```python
from build123d import *

# Parameters (mm, degrees)
SKETCH_1_R               = 210
EXTRUDE_1_DEPTH          = 25
SKETCH_2_R               = 95.82
CUT_EXTRUDE_1_DEPTH      = 154
EXTRUDE_START            = 200
SKETCH_3_R               = 155.82
SKETCH_3_R_2             = 95.82
EXTRUDE_2_DEPTH          = 200
CHAMFER_1_SIZE           = 1
SKETCH_7_R               = 140.82
SKETCH_7_R_2             = 105.82
CUT_EXTRUDE_3_DEPTH      = 200
PATTERN_CIRCULAR_2_COUNT = 8


with BuildPart() as part:
    # 草图1 → 凸台-拉伸1 (new body)
    with BuildSketch(Plane(origin=(0, 0, 0), x_dir=(1, 0, 0), z_dir=(0, 1, 0))):
        with Locations(Location((0, 0, 0), (0, 0, 270))):
            Circle(SKETCH_1_R)
    extrude(amount=EXTRUDE_1_DEPTH)

    # 草图2 → 切除-拉伸1 (cut)
    with BuildSketch(Plane(origin=(0, 25, 0), x_dir=(1, 0, 0), z_dir=(0, 1, 0))):
        with Locations(Location((0, 0, 0), (0, 0, 270))):
            Circle(SKETCH_2_R)
    extrude(amount=-CUT_EXTRUDE_1_DEPTH, mode=Mode.SUBTRACT)

    # 草图3 → 凸台-拉伸2 (add)
    with BuildSketch(Plane(origin=(0, 25, 0), x_dir=(1, 0, 0), z_dir=(0, 1, 0)).offset(EXTRUDE_START)):
        with Locations(Location((0, 0, 0), (0, 0, 270))):
            Circle(SKETCH_3_R)
        with Locations(Location((0, 0, 0), (0, 0, 270))):
            Circle(SKETCH_3_R_2, mode=Mode.SUBTRACT)
    extrude(amount=-EXTRUDE_2_DEPTH)

    # 倒角1
    chamfer_1_edges = [part.edges().sort_by_distance(p)[0] for p in [
        (0, 225, -155.82),
        (0, 225, -95.82),
        (0, 0, -210),
        (0, 25, -210),
    ]]
    chamfer(chamfer_1_edges, length=CHAMFER_1_SIZE)

    # 草图7 → 切除-拉伸3 (cut)
    with BuildSketch(Plane(origin=(0, 225, 0), x_dir=(1, 0, 0), z_dir=(0, 1, 0))):
        with Locations(Location((0, 0, 0), (0, 0, 270))):
            Circle(SKETCH_7_R)
        with Locations(Location((0, 0, 0), (0, 0, 270))):
            Circle(SKETCH_7_R_2, mode=Mode.SUBTRACT)
    extrude(amount=-CUT_EXTRUDE_3_DEPTH, mode=Mode.SUBTRACT)

    # 草图10 → M10 六角圆柱头螺钉的柱形沉头孔2 (revolve, cut)
    with BuildSketch(Plane(origin=(-184.987401502, 25, 2.159001035), x_dir=(0, 0, 1), z_dir=(1, 0, 0))):
        Polygon((0, 0), (0, 30.804733405), (5.5, 27.5), (5.5, 11), (9, 11), (9, 0.025), (9.025, 0), align=None)
    hole_wizard_m10_2 = revolve(axis=Axis((-184.987401502, 31.35, 2.159001035), (0, -1, 0)), mode=Mode.SUBTRACT)

    # 阵列(圆周)2: M10 六角圆柱头螺钉的柱形沉头孔2 ×8 about axis
    pattern_circular_2_axis = Axis((0, 0, 0), (0, 1, 0))
    for i in range(1, PATTERN_CIRCULAR_2_COUNT):
        add(hole_wizard_m10_2.rotate(pattern_circular_2_axis, i * 360 / PATTERN_CIRCULAR_2_COUNT), mode=Mode.SUBTRACT)


solid = part.part
```
Source: CAD feature listing. Evaluate the final solid. Frame: model axes, mm. A direction names the side the tool comes from. Give positions to 0.01 mm unless a question says otherwise; leave off trailing zeros. Order: outer loops, then holes, each group sorted by start corner. A loop starts at its lowest first (then second) coordinate and runs counter-clockwise, first axis right, second up. Notation, with made-up numbers: (78.25, 75.25) -> (111.25, 75.25) arc R25 cw to (111.25, 112.25) -> close; hole circle Ø11 at (77, -22.75). An arc over 180 degrees is marked (long way). Use a Markdown table: item, result.
Q1. Section A-A (y = 104). Return the cut outline in (x, z), and give its area (3 significant figures).
A:
| item | result |
|---|---|
| outline | circle Ø311.64 at (0, 0); circle Ø211.64 at (0, 0); hole circle Ø281.64 at (0, 0); hole circle Ø191.64 at (0, 0) |
| area | 20,300 mm^2 |
Q2. First-contact query: P1, Ø2, axis at y = 38.5, z = 98.5, coming from the +X side; P2, Ø1.5, axis at x = 95.5, y = 145, coming from the -Z side; P3, Ø17.5, axis at x = 129.28, z = -132.33, coming from the +Y side; P4, Ø9, axis at x = -2.16, z = -184.99, coming from the +Y side. Flat tips, straight axial feed; report the tip coordinate or a pass-through.
A:
| item | result |
|---|---|
| P1 | x = 121.55 |
| P2 | z = -123.7 |
| P3 | y = 14 |
| P4 | through |
Q3. Pull-direction query (X, two-part tool) for faces 3 (the face through (63.08, 12.34, 200.3)), 4 (the face through (-86, 225, 47)), 5 (the face through (-137.81, 19.56, -136.42)); classes: +X half, -X half, draft (parallel to the pull), parting line (faces both ways), or undercut.
A:
| item | result |
|---|---|
| face 3 | parting line |
| face 4 | draft |
| face 5 | undercut |
Q4. Access query for faces 1 (the face through (-132.095, 7.098, -134.774)), 2 (the face through (125, 25, -94)). Directions: +Z, -Z, +X, -X, +Y, -Y. A direction counts if a zero-diameter tool reaches every point of the face in a straight line with its end or side. Return the directions, or none.
A:
| item | result |
|---|---|
| face 1 | +Y, -Y |
| face 2 | +Y |
Q5. Material intervals for line 1 (Z direction, x = 37.5, y = 34.5); line 2 (Z direction, x = -12, y = 30); line 3 (X direction, y = 195, z = -17), sorted ascending. Write a range as [from, to].
A:
| item | result |
|---|---|
| line 1 | [-151.24, -135.74], [-98.95, -88.18], [88.18, 98.95], [135.74, 151.24] |
| line 2 | [-155.36, -140.31], [-105.14, -95.07], [95.07, 105.14], [140.31, 155.36] |
| line 3 | [-154.89, -139.79], [-104.45, -94.3], [94.3, 104.45], [139.79, 154.89] |
